For this review, take the finished solid that the model builds, in its own axes (mm). Face numbers are marked on the shaded views. A direction names the side the tool comes from. Coordinates: 2 decimals unless noted, no trailing zeros. Loops run counter-clockwise (first coordinate to the right, second up) from the corner with the lowest first, then second, coordinate; pieces in that order, holes last.
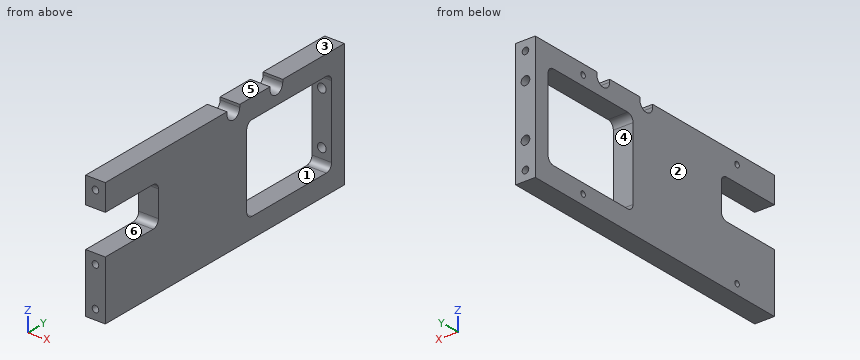
```python
from build123d import *

# Parameters (mm, degrees)
SKETCH1_W                  = 95
SKETCH1_H                  = 225.1
BOSS_EXTRUDE1_DEPTH        = 15
CUT_EXTRUDE1_DEPTH         = 124.080268524
M6_CLEARANCE_HOLE1_D       = 6.6
M6_CLEARANCE_HOLE1_DEPTH   = 19.75
M6_CLEARANCE_HOLE1_TIP     = 1.982840043
M6_TAPPED_HOLE1_D          = 5
M6_TAPPED_HOLE1_DEPTH      = 15
M6_TAPPED_HOLE1_TIP        = 1.502151548
F_5_0MM_BLIND_HOLE_1_D     = 5
F_5_0MM_BLIND_HOLE_1_DEPTH = 8
F_5_0MM_BLIND_HOLE_1_TIP   = 1.502151548
F_5_0MM_BLIND_HOLE_2_D     = 5
F_5_0MM_BLIND_HOLE_2_DEPTH = 8
F_5_0MM_BLIND_HOLE_2_TIP   = 1.502151548
SKETCH14_R                 = 6
CUT_EXTRUDE2_DEPTH         = 124.080268524
SKETCH15_W                 = 10
SKETCH15_H                 = 12
CUT_EXTRUDE3_DEPTH         = 124.080268524
M5_TAPPED_HOLE1_AT_2_COUNT = 2
M5_TAPPED_HOLE1_AT_2_PITCH = 145


with BuildPart() as part:
    # Sketch1 → Boss-Extrude1 (new body)
    with BuildSketch(Plane(origin=(0, 0, 0), x_dir=(0, 0, -1), z_dir=(1, 0, 0))):
        Rectangle(SKETCH1_W, SKETCH1_H)
    extrude(amount=BOSS_EXTRUDE1_DEPTH)

    # Sketch2 → Cut-Extrude1 (cut, through all)
    with BuildSketch(Plane.ZY):
        with BuildLine():
            Line((22.5, -62.55), (2.5, -62.55))
            ThreePointArc((2.5, -62.55), (-1.035533906, -64.014466094), (-2.5, -67.55))
            Line((-2.5, -67.55), (-2.5, -112.55))
            Line((-2.5, -112.55), (27.5, -112.55))
            Line((27.5, -112.55), (27.5, -67.55))
            ThreePointArc((27.5, -67.55), (26.035533906, -64.014466094), (22.5, -62.55))
        make_face()
        with BuildLine():
            Line((-27.5, 20.55), (27.5, 20.55))
            ThreePointArc((27.5, 20.55), (31.035533906, 22.014466094), (32.5, 25.55))
            Line((32.5, 25.55), (32.5, 95.55))
            ThreePointArc((32.5, 95.55), (31.035533906, 99.085533906), (27.5, 100.55))
            Line((27.5, 100.55), (-27.5, 100.55))
            ThreePointArc((-27.5, 100.55), (-31.035533906, 99.085533906), (-32.5, 95.55))
            Line((-32.5, 95.55), (-32.5, 25.55))
            ThreePointArc((-32.5, 25.55), (-31.035533906, 22.014466094), (-27.5, 20.55))
        make_face()
    extrude(amount=-CUT_EXTRUDE1_DEPTH, mode=Mode.SUBTRACT)

    # M6 Clearance Hole1
    with Locations(Plane(origin=(0, 112.55, 0), x_dir=(1, 0, 0), z_dir=(0, 1, 0))):
        with Locations((7.5, -20), (7.5, 20)):
            Hole(M6_CLEARANCE_HOLE1_D / 2, depth=M6_CLEARANCE_HOLE1_DEPTH)
            with Locations((0, 0, -(M6_CLEARANCE_HOLE1_DEPTH + M6_CLEARANCE_HOLE1_TIP / 2))):  # 118° drill point
                Cone(0, M6_CLEARANCE_HOLE1_D / 2, M6_CLEARANCE_HOLE1_TIP, mode=Mode.SUBTRACT)

    # M6 Tapped Hole1
    with Locations(Plane(origin=(0, -112.55, 0), x_dir=(-1, 0, 0), z_dir=(0, -1, 0))):
        with Locations((-7.5, -40), (-7.5, 40)):
            Hole(M6_TAPPED_HOLE1_D / 2, depth=M6_TAPPED_HOLE1_DEPTH)
            with Locations((0, 0, -(M6_TAPPED_HOLE1_DEPTH + M6_TAPPED_HOLE1_TIP / 2))):  # 118° drill point
                Cone(0, M6_TAPPED_HOLE1_D / 2, M6_TAPPED_HOLE1_TIP, mode=Mode.SUBTRACT)

    # Ø5.0mm blind hole 1
    with Locations(Plane(origin=(0, -112.55, 0), x_dir=(-1, 0, 0), z_dir=(0, -1, 0))):
        with Locations((-7.5, 10)):
            Hole(F_5_0MM_BLIND_HOLE_1_D / 2, depth=F_5_0MM_BLIND_HOLE_1_DEPTH)
            with Locations((0, 0, -(F_5_0MM_BLIND_HOLE_1_DEPTH + F_5_0MM_BLIND_HOLE_1_TIP / 2))):  # 118° drill point
                Cone(0, F_5_0MM_BLIND_HOLE_1_D / 2, F_5_0MM_BLIND_HOLE_1_TIP, mode=Mode.SUBTRACT)

    # Ø5.0mm blind hole 2
    with Locations(Plane(origin=(0, 112.55, 0), x_dir=(1, 0, 0), z_dir=(0, 1, 0))):
        with Locations((7.5, -40), (7.5, 40)):
            Hole(F_5_0MM_BLIND_HOLE_2_D / 2, depth=F_5_0MM_BLIND_HOLE_2_DEPTH)
            with Locations((0, 0, -(F_5_0MM_BLIND_HOLE_2_DEPTH + F_5_0MM_BLIND_HOLE_2_TIP / 2))):  # 118° drill point
                Cone(0, F_5_0MM_BLIND_HOLE_2_D / 2, F_5_0MM_BLIND_HOLE_2_TIP, mode=Mode.SUBTRACT)

    # Sketch14 → Cut-Extrude2 (cut, through all)
    with BuildSketch(Plane(origin=(15, 0, 0), x_dir=(0, 0, -1), z_dir=(1, 0, 0))):
        with Locations((-45.5, 48.55)):
            Circle(SKETCH14_R)
        with Locations((-45.5, 8.05)):
            Circle(SKETCH14_R)
    extrude(amount=-CUT_EXTRUDE2_DEPTH, mode=Mode.SUBTRACT)

    # Sketch15 → Cut-Extrude3 (cut, through all)
    with BuildSketch(Plane.ZY):
        with Locations((50.5, 8.05)):
            Rectangle(SKETCH15_W, SKETCH15_H)
        with Locations((50.5, 48.55)):
            Rectangle(SKETCH15_W, SKETCH15_H)
    extrude(amount=-CUT_EXTRUDE3_DEPTH, mode=Mode.SUBTRACT)

    # Sketch19 → M5 Tapped Hole1 (revolve, cut)
    with BuildSketch(Plane(origin=(0, -77.45, -40), x_dir=(0, 0, 1), z_dir=(0, 1, 0))):
        Polygon((0, 0), (0, 13.6618073), (2.1, 12.4), (2.1, 0), align=None)
    m5_tapped_hole1 = revolve(axis=Axis((-6.35, -77.45, -40), (1, 0, 0)), mode=Mode.SUBTRACT)

    # M5 Tapped Hole1 at 2: M5 Tapped Hole1 ×2
    with Locations(*[(0, i * M5_TAPPED_HOLE1_AT_2_PITCH, 0) for i in range(1, M5_TAPPED_HOLE1_AT_2_COUNT)]):
        add(m5_tapped_hole1, mode=Mode.SUBTRACT)

    # Mirror1: M5 Tapped Hole1 across plane
    add(m5_tapped_hole1.mirror(Plane.XY), mode=Mode.SUBTRACT)

    # Mirror1 copy 1 sketch → Mirror1 copy 1 (revolve, cut)
    with BuildSketch(Plane(origin=(0, 67.55, 40), x_dir=(0, 0, -1), z_dir=(0, 1, 0))):
        Polygon((0, 0), (0, -13.6618073), (2.1, -12.4), (2.1, 0), align=None)
    revolve(axis=Axis((-6.35, 67.55, 40), (-1, 0, 0)), mode=Mode.SUBTRACT)


solid = part.part
```
Q1. Consider section C-C (y = 8.05). State the section outline as (x, z) points.
Q2. Machinability: for the marked faces 4, 5 and 6, which of the approach directions +Z, -Z, +X, -X, +Y, -Y give a long, thin tool a straight path to every point of the face, cutting with its end or side? Answer none if there is none.
Q3. The part is to be moulded in two halves that separate along Z. For the marked faces 1, 2 and 3, say which applies: +Z half, -Z half, draft (parallel to the pull), parting line (faces both ways), or undercut.
Q4. For pin 1 Ø4.5 at (x, z) = (7.5, -40) entering from -Y; pin 2 Ø4 at (y, z) = (67.55, 40) entering from -X, all flat-tipped, find the tip position at first contact; note any pin that passes through.
Q5. Consider section A-A (y = 48.55). State the section outline as (x, z) points.
Q6. Wall thickness on probe 1 along Z at (x, y) = (7.5, 108.25); probe 2 along Y at (x, z) = (3.5, -40); probe 3 along Z at (x, y) = (7.5, -101.5): over which ranges is each line inside the solid? List them lowest first.
Q7. Consider section B-B (y = -88.5). State the section outline as (x, z) points, then the cut area to 3 significant figures.
Model answer:
1. outline: (0, -47.5) - (15, -47.5) - (15, 39.5) - (0, 39.5) - close
2. face 4: +X, -X
2. face 5: +Z, +X, -X, +Y, -Y
2. face 6: +X, -X, -Y
3. face 1: undercut
3. face 2: draft
3. face 3: +Z half
4. pin 1: stops at y = -97.4
4. pin 2: stops at x = 12.46
5. outline: (0, -47.5) - (15, -47.5) - (15, -32.5) - (0, -32.5) - close; (0, 32.5) - (15, 32.5) - (15, 39.5) - (0, 39.5) - close
6. probe 1: z = -47.5 to -42.5, -37.5 to -23.3, -16.7 to 16.7, 23.3 to 37.5, 42.5 to 47.5
6. probe 2: y = -112.55 to -79.55, -75.35 to 65.45, 69.65 to 112.55
6. probe 3: z = -47.5 to -42.5, -37.5 to -2.5, 27.5 to 37.5, 42.5 to 47.5
7. outline: (0, -47.5) - (15, -47.5) - (15, -2.5) - (0, -2.5) - close; (0, 27.5) - (15, 27.5) - (15, 47.5) - (0, 47.5) - close
7. area: 975 mm2
